from build123d import *

# Parameters (mm, degrees)
SKETCH1_R             = 32.5
SKETCH1_R_2           = 31.5
BOSS_EXTRUDE1_DEPTH   = 6
SKETCH1_R_3           = 28.5
SKETCH1_R_4           = 27.5
BOSS_EXTRUDE1_2_DEPTH = 6
SKETCH2_R             = 34.5
SKETCH2_R_2           = 27.5
BOSS_EXTRUDE2_DEPTH   = 1.2


with BuildPart() as part:
    # Sketch1 → Boss-Extrude1 (new body)
    with BuildSketch(Plane.XY):
        Circle(SKETCH1_R)
        Circle(SKETCH1_R_2, mode=Mode.SUBTRACT)
    extrude(amount=BOSS_EXTRUDE1_DEPTH)



with BuildPart() as body_2:
    # Sketch1 → Boss-Extrude1 2 (new body)
    with BuildSketch(Plane.XY):
        Circle(SKETCH1_R_3)
        Circle(SKETCH1_R_4, mode=Mode.SUBTRACT)
    extrude(amount=BOSS_EXTRUDE1_2_DEPTH)


with BuildPart() as part_1:
    add(part.part)

    add(body_2.part)  # Boss-Extrude2 merges body 2
    # Sketch2 → Boss-Extrude2 (add)
    with BuildSketch(Plane.XY):
        Circle(SKETCH2_R)
        Circle(SKETCH2_R_2, mode=Mode.SUBTRACT)
    extrude(amount=BOSS_EXTRUDE2_DEPTH)


solid = part_1.part
Source: CAD feature listing. Evaluate the final solid. Frame: model axes, mm. A direction names the side the tool comes from. Give positions to 0.01 mm unless a question says otherwise; leave off trailing zeros. Write each loop counter-clockwise with the first axis right and the second up, starting at its lowest first coordinate (ties: lowest second). Pieces come first, ordered by that corner, then holes. Notation, with made-up numbers: M -7.5,61 L 41.5,61 A22 ccw 41.5,78 Z; hole C 70.5,12 d9. An arc over 180 degrees is marked long. Return JSON: item names as keys, results as strings. Group by question number.
1) Cut plane C-C, the plane z = 2.45. Output: boundary loops of the cut face in (x, y), then the cut area to 3 significant figures.
2) First-contact query: pin 1 Ø1.5 at (x, z) = (9, 3.5) entering from -Y; pin 2 Ø1 at (x, y) = (17.5, 25.5) entering from -Z; pin 3 Ø2 at (y, z) = (-3, 2.5) entering from -X; pin 4 Ø1 at (x, z) = (-1.5, 2) entering from +Y. Flat tips, straight axial feed; report the tip coordinate or a pass-through.
3) Cut plane A-A, the plane y = 0. Output: boundary loops of the cut face in (x, z), then the cut area to 3 significant figures.
4) Draft query along Y for faces 3 (the face through (-4.101, 31.232, 3.566)), 4 (the face through (-23.2, -15.2, 0)), 5 (the face through (32.907, 10.363, 0.592)). Return one class per face: released by +Y, released by -Y, zero draft, split by the parting line, or undercut.
5) Set-up query: faces 1 (the face through (31, 9.76, 3.57)), 2 (the face through (-17, 27, 6)). Return all of +Z, -Z, +X, -X, +Y, -Y with unobstructed straight access to the full face (end or side cutting, diameter ignored); none if empty.
6) Cut plane B-B, the plane x = -8.5. Output: boundary loops of the cut face in (y, z).
7) Ray query, L1, parallel to Y at x = 0, z = 5.05; L2, parallel to Y at x = 6, z = 5.15; L3, parallel to X at y = -18, z = 1.7. Return the intervals inside material, ascending.
Data:
{
 "1": {"outline": "C 0,0 d65; C 0,0 d57; hole C 0,0 d63; hole C 0,0 d55", "area": "377 mm²"},
 "2": {"pin 1": "stops at y = -31.44", "pin 2": "stops at z = 0", "pin 3": "stops at x = -32.44", "pin 4": "stops at y = 32.48"},
 "3": {"outline": "M -34.5,0 L -27.5,0 L -27.5,6 L -28.5,6 L -28.5,1.2 L -31.5,1.2 L -31.5,6 L -32.5,6 L -32.5,1.2 L -34.5,1.2 Z; M 27.5,0 L 34.5,0 L 34.5,1.2 L 32.5,1.2 L 32.5,6 L 31.5,6 L 31.5,1.2 L 28.5,1.2 L 28.5,6 L 27.5,6 Z", "area": "36.0 mm²"},
 "4": {"face 3": "undercut", "face 4": "zero draft", "face 5": "split by the parting line"},
 "5": {"face 1": "+Z", "face 2": "+Z, +X, -X, +Y, -Y"},
 "6": {"outline": "M -33.44,0 L -26.15,0 L -26.15,6 L -27.2,6 L -27.2,1.2 L -30.33,1.2 L -30.33,6 L -31.37,6 L -31.37,1.2 L -33.44,1.2 Z; M 26.15,0 L 33.44,0 L 33.44,1.2 L 31.37,1.2 L 31.37,6 L 30.33,6 L 30.33,1.2 L 27.2,1.2 L 27.2,6 L 26.15,6 Z"},
 "7": {"L1": "y = -32.5 to -31.5, -28.5 to -27.5, 27.5 to 28.5, 31.5 to 32.5", "L2": "y = -31.94 to -30.92, -27.86 to -26.84, 26.84 to 27.86, 30.92 to 31.94", "L3": "x = -27.06 to -25.85, -22.1 to -20.79, 20.79 to 22.1, 25.85 to 27.06"}
}
